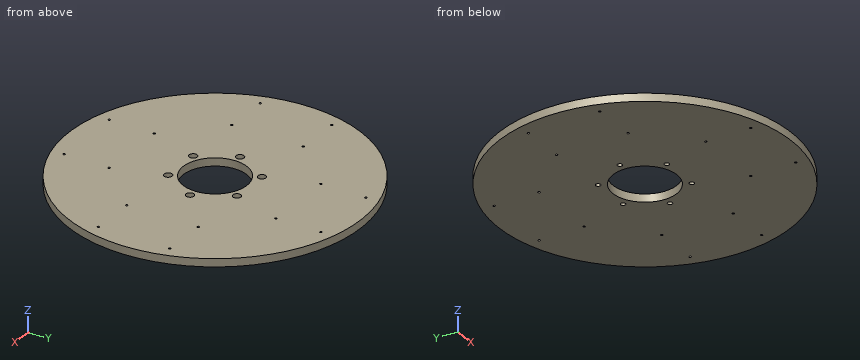
```python
from build123d import *

# Parameters (mm, degrees)
SKETCH1_R                                         = 275
BOSS_EXTRUDE1_DEPTH                               = 15
SKETCH2_R                                         = 60
CUT_EXTRUDE1_DEPTH                                = 390.197893108
M5_TAPPED_HOLE1_D                                 = 4.2
CIRPATTERN1_COUNT                                 = 4
HOLE_SIZE_BASED_SOCKET_HEAD_CAP_SCREW_D           = 9
HOLE_SIZE_BASED_SOCKET_HEAD_CAP_SCREW_CBORE_D     = 15
HOLE_SIZE_BASED_SOCKET_HEAD_CAP_SCREW_CBORE_DEPTH = 9
CIRPATTERN2_COUNT                                 = 6


with BuildPart() as part:
    # Sketch1 → Boss-Extrude1 (new body)
    with BuildSketch(Plane.XY):
        Circle(SKETCH1_R)
    extrude(amount=BOSS_EXTRUDE1_DEPTH)

    # Sketch2 → Cut-Extrude1 (cut, through all)
    with BuildSketch(Plane.XY.offset(15)):
        Circle(SKETCH2_R)
    extrude(amount=-CUT_EXTRUDE1_DEPTH, mode=Mode.SUBTRACT)

    # M5 Tapped Hole1 (through all)
    with Locations(Plane.XY.offset(15)):
        with Locations((67.5, 157.5), (67.5, 242.5), (-67.5, 157.5), (-67.5, 242.5)):
            m5_tapped_hole1 = Hole(M5_TAPPED_HOLE1_D / 2)

    # CirPattern1: M5 Tapped Hole1 ×4 about axis
    cirpattern1_axis = Axis((0, 0, 0), (0, 0, 1))
    for i in range(1, CIRPATTERN1_COUNT):
        add(m5_tapped_hole1.rotate(cirpattern1_axis, i * 360 / CIRPATTERN1_COUNT), mode=Mode.SUBTRACT)

    # Hole Size (%based) Socket Head Cap Screw Type1 (through all)
    with Locations(Plane.XY.offset(15)):
        with Locations((-37.5, 64.951905284)):
            hole_size_based_socket_head_cap_screw = CounterBoreHole(HOLE_SIZE_BASED_SOCKET_HEAD_CAP_SCREW_D / 2, HOLE_SIZE_BASED_SOCKET_HEAD_CAP_SCREW_CBORE_D / 2, HOLE_SIZE_BASED_SOCKET_HEAD_CAP_SCREW_CBORE_DEPTH)

    # CirPattern2: Hole Size (%based) Socket Head Cap Screw Type1 ×6 about axis
    cirpattern2_axis = Axis((0, 0, 0), (0, 0, 1))
    for i in range(1, CIRPATTERN2_COUNT):
        add(hole_size_based_socket_head_cap_screw.rotate(cirpattern2_axis, i * 360 / CIRPATTERN2_COUNT), mode=Mode.SUBTRACT)


solid = part.part
```
Design review of the part built by this model. Coordinates are the model's own, in mm. Coordinates: 2 decimals unless noted, no trailing zeros. Order: outer loops, then holes, each group sorted by start corner. A loop starts at its lowest first (then second) coordinate and runs counter-clockwise, first axis right, second up.
1) Take a section at B-B, the plane x = 8.5. Give the boundary of the cut face in (y, z), and give its area (3 significant figures).
2) Wall thickness on line 1 along Y through (x, z) = (-242.5, 10.75); line 2 along Y through (x, z) = (-37.5, 2.5): over which ranges is each line inside the solid? List them lowest first.
3) Take a section at D-D, the plane y = 227. Give the boundary of the cut face in (x, z), and give its area (3 significant figures).
4) Clearance check with flat-ended pins moving along their axes: pin 1 (3.5 mm diameter, centred on x = 67.5, y = -157.5, fed in from -Z); pin 2 (7.5 mm diameter, centred on x = 75, y = 1.5, fed in from +Z); pin 3 (2 mm diameter, centred on x = 38, z = 9, fed in from -Y); pin 4 (8 mm diameter, centred on y = 202, z = 5.5, fed in from -X). State where each tip first meets the part, or that it passes through.
5) Take a section at A-A, the plane y = -40.5. Give the boundary of the cut face in (x, z), and give its area (3 significant figures).
6) Take a section at C-C, the plane z = 8.5. State how many separate pieces and enclosed holes the cut face has, and give its area (3 significant figures).
Returned:
1. outline: (-274.87, 0) - (-59.39, 0) - (-59.39, 15) - (-274.87, 15) - close; (59.39, 0) - (274.87, 0) - (274.87, 15) - (59.39, 15) - close
1. area: 6,460 mm2
2. line 1: y = -129.69 to -69.6, -65.4 to 65.4, 69.6 to 129.69
2. line 2: y = -272.43 to -69.45, -60.45 to -46.84, 46.84 to 60.45, 69.45 to 272.43
3. outline: (-155.23, 0) - (155.23, 0) - (155.23, 15) - (-155.23, 15) - close
3. area: 4,660 mm2
4. pin 1: passes through
4. pin 2: stops at z = 6
4. pin 3: stops at y = -272.5
4. pin 4: stops at x = -190.84
5. outline: (-272, 0) - (-44.27, 0) - (-44.27, 15) - (-272, 15) - close; (44.27, 0) - (272, 0) - (272, 15) - (44.27, 15) - close
5. area: 6,830 mm2
6. separate pieces: 1
6. enclosed holes: 23
6. area: 225,000 mm2
